Model file for the job. Use its own axes, mm. A direction names the side the tool comes from. Round coordinates to 2 decimals unless told otherwise and drop trailing zeros. Write each loop counter-clockwise with the first axis right and the second up, starting at its lowest first coordinate (ties: lowest second). Pieces come first, ordered by that corner, then holes. Notation, with made-up numbers: (67, -31.75) - (88, -31.75) arc R28 ccw to (88, -10.75) - close; hole circle Ø10 at (-37, 83.5). An arc over 180 degrees is marked (long way). Answer as a JSON object with one key per item and string values. Group by question number.
from build123d import *

# Parameters (mm, degrees)
SKETCH_1_W                = 40
SKETCH_1_H                = 32
EXTRUDE_1_DEPTH           = 8
SKETCH_8_R                = 6
CUT_EXTRUDE_2_DEPTH       = 27.83281573
HOLE_WIZARD_3_D           = 5.5
HOLE_WIZARD_3_CBORE_D     = 10
HOLE_WIZARD_3_CBORE_DEPTH = 5.7
HOLE_WIZARD_M5_1_D        = 4.2
HOLE_WIZARD_M5_1_DEPTH    = 12.4
HOLE_WIZARD_M5_1_TIP      = 1.2618073


with BuildPart() as part:
    # 草图1 → 凸台-拉伸1 (new body)
    with BuildSketch(Plane(origin=(0, 0, 0), x_dir=(0, 0, -1), z_dir=(1, 0, 0))):
        Rectangle(SKETCH_1_W, SKETCH_1_H)
    extrude(amount=EXTRUDE_1_DEPTH)

    # 草图8 → 切除-拉伸2 (cut, through all)
    with BuildSketch(Plane.ZY):
        with Locations((3.523652159, 0)):
            Circle(SKETCH_8_R)
    extrude(amount=-CUT_EXTRUDE_2_DEPTH, mode=Mode.SUBTRACT)

    # 打孔尺寸(%根据)内六角圆柱头螺钉的类型3 (through all)
    with Locations(Plane.ZY):
        with Locations((-6.375842777, 9.899494937), (13.423147096, -9.899494937)):
            CounterBoreHole(HOLE_WIZARD_3_D / 2, HOLE_WIZARD_3_CBORE_D / 2, HOLE_WIZARD_3_CBORE_DEPTH)

    # M5 螺纹孔1
    with Locations(Plane(origin=(0, 16, 0), x_dir=(1, 0, 0), z_dir=(0, 1, 0))):
        with Locations((4, -3), (4, -15), (4, 15)):
            Hole(HOLE_WIZARD_M5_1_D / 2, depth=HOLE_WIZARD_M5_1_DEPTH)
            with Locations((0, 0, -(HOLE_WIZARD_M5_1_DEPTH + HOLE_WIZARD_M5_1_TIP / 2))):  # 118° drill point
                Cone(0, HOLE_WIZARD_M5_1_D / 2, HOLE_WIZARD_M5_1_TIP, mode=Mode.SUBTRACT)


solid = part.part
(1) Slice it at C-C (y = -10.5). Write the cut outline in (x, z), then the cut area to 3 significant figures.
(2) Pull direction Y, two halves, no side cores. Call faces 1 (the cylindrical face through (2.81, 7.98, -1.76)), 2 (the flat face through (5.7, 8, -4)), 3 (the flat face through (0, 0, -4)), 4 (the conical face through (3.953, 2.557, 14.638)): pulls with the +Y half, pulls with the -Y half, needs draft (parallel to the pull), parting line crosses it, or undercut.
(3) Slice it at A-A (y = 8). Write the cut outline in (x, z), then the cut area to 3 significant figures.
(4) Slice it at B-B (x = 7). Write the cut outline in (y, z), then the cut area to 3 significant figures.
(5) Slice it at D-D (x = 4.5). Count the separate pieces of the cut face and the enclosed holes in it, then the cut area to 3 significant figures.
(6) Flat gauge pins, fed straight in: pin 1 (3.5 mm diameter, centred on x = 4, z = 3, fed in from +Y); pin 2 (7 mm diameter, centred on y = 0, z = 3.52, fed in from -X); pin 3 (6 mm diameter, centred on y = -9.9, z = 13.42, fed in from +X); pin 4 (5 mm diameter, centred on y = 8, z = -7.5, fed in from -X). Where does each tip first touch, or does it go through?
(7) Drill centre lines: line 1 (Z direction, x = 4, y = 12.75); line 2 (X direction, y = 12, z = 15); line 3 (Z direction, x = 5.75, y = -10). Where is each one in solid material? Low to high. Write a range as from..to.
(8) 3-axis set-ups, long thin cutter, end or side, ignore diameter. For faces 5 (the cylindrical face through (6.866, -12.339, 12.154)), 6 (the flat face through (5.7, -12, 16)), 7 (the cylindrical face through (2.87, 10.62, 1.23)): which of +Z, -Z, +X, -X, +Y, -Y reach the whole face in a straight line?
Answer:
{
 "1": {"outline": "(0, -20) - (8, -20) - (8, 10.74) - (5.7, 10.74) - (5.7, 8.46) - (0, 8.46) - close; (0, 18.39) - (5.7, 18.39) - (5.7, 16.11) - (8, 16.11) - (8, 20) - (0, 20) - close", "area": "251 mm²"},
 "2": {"face 1": "undercut", "face 2": "undercut", "face 3": "needs draft", "face 4": "pulls with the +Y half"},
 "3": {"outline": "(0, -20) - (8, -20) - (8, -8.36) - (5.7, -8.36) - (5.7, -11) - (0, -11) - close; (0, -1.75) - (5.7, -1.75) - (5.7, -4.39) - (8, -4.39) - (8, 20) - (0, 20) - close; hole circle Ø4.2 at (4, -15); hole circle Ø4.2 at (4, 3); hole circle Ø4.2 at (4, 15)", "area": "217 mm²"},
 "4": {"outline": "(-16, -20) - (16, -20) - (16, 20) - (-16, 20) - close; hole circle Ø5.5 at (-9.9, 13.42); hole circle Ø12 at (0, 3.52); hole circle Ø5.5 at (9.9, -6.38)", "area": "1,120 mm²"},
 "5": {"separate pieces": "1", "enclosed holes": "2", "area": "863 mm²"},
 "6": {"pin 1": "y = -5.55", "pin 2": "through", "pin 3": "x = 8", "pin 4": "x = 5.7"},
 "7": {"line 1": "-20..-17.1, -12.9..-10.48, -2.27..0.9, 5.1..12.9, 17.1..20", "line 2": "0..1.9, 6.1..8", "line 3": "-20..10.67, 16.17..20"},
 "8": {"face 5": "+X, -X", "face 6": "-X", "face 7": "+Y"}
}
